Here's how the part is built. I have some questions about the finished solid (model axes, mm). Face numbers are marked on the shaded views. A direction names the side the tool comes from. Give positions to 0.01 mm unless a question says otherwise; leave off trailing zeros. Loops run counter-clockwise (first coordinate to the right, second up) from the corner with the lowest first, then second, coordinate; pieces in that order, holes last.
Q1. Suppose I cut it at B-B (z = 0). List the corners of the cut face in (x, y) for me.
Q2. Suppose I cut it at C-C (y = 7). List the corners of the cut face in (x, z) for me, and give its area (3 significant figures).
Q3. Suppose I cut it at D-D (y = 37). List the corners of the cut face in (x, z) for me, and give its area (3 significant figures).
Q4. I'm going to push flat-ended pins straight in: P1, Ø5, axis at y = 19, z = 3, coming from the +X side; P2, Ø6, axis at x = -1, y = 27.5, coming from the +Z side; P3, Ø2, axis at y = 16.5, z = -1.5, coming from the -X side. Where does each tip first touch, or does it pass through?
Q5. For the marked faces 1 and 2, which set-ups out of +Z, -Z, +X, -X, +Y, -Y let a thin tool reach every point of the face, with its end or its side?
Q6. Suppose I cut it at A-A (x = 0). List the corners of the cut face in (y, z) for me.
Q7. I need wall thicknesses on probe 1 along Y at (x, z) = (-5.75, 2); probe 2 along X at (y, z) = (27, -3); probe 3 along X at (y, z) = (12, 0.25). Which ranges of each line are inside material? Lowest first, please.
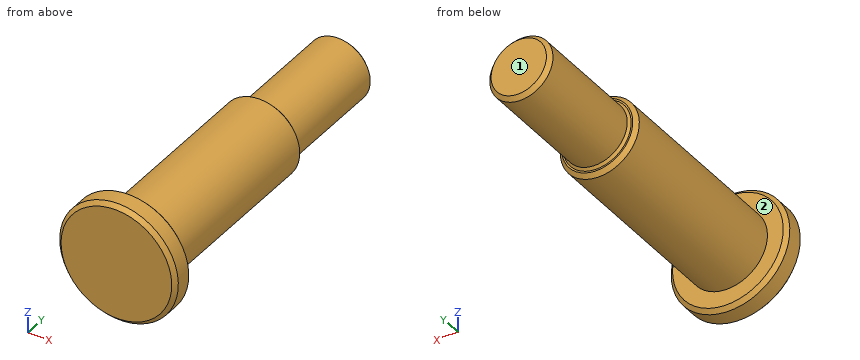
```python
from build123d import *

# Parameters (mm, degrees)
CHAMFER1_SIZE = 0.5
CHAMFER2_SIZE = 0.3


with BuildPart() as part:
    # Sketch1 → Revolve1 (revolve)
    with BuildSketch(Plane.XY, mode=Mode.PRIVATE) as revolve1_sk:
        Polygon((0, 0), (7.5, 0), (7.5, 3), (5, 3), (5, 28), (4, 28), (4, 43), (0, 43), align=None)
    revolve(revolve1_sk.sketch.rotate(Axis((0, 0, 0), (0, -1, 0)), 90), axis=Axis((0, 0, 0), (0, -1, 0)))

    # Chamfer1
    chamfer1_edges = [part.edges().sort_by_distance(p)[0] for p in [
        (0, 43, -4),
        (0, 28, -5),
        (0, 3, -7.5),
        (0, 0, -7.5),
    ]]
    chamfer(chamfer1_edges, length=CHAMFER1_SIZE)

    # Chamfer2
    chamfer2_edges = [part.edges().sort_by_distance(p)[0] for p in [
        (0, 28, -4),
    ]]
    chamfer(chamfer2_edges, length=CHAMFER2_SIZE)


solid = part.part
```
Solutions:
1. outline: (-7.5, 0.5) - (-7, 0) - (7, 0) - (7.5, 0.5) - (7.5, 2.5) - (7, 3) - (5, 3) - (5, 27.5) - (4.5, 28) - (4.3, 28) - (4, 28.3) - (4, 42.5) - (3.5, 43) - (-3.5, 43) - (-4, 42.5) - (-4, 28.3) - (-4.3, 28) - (-4.5, 28) - (-5, 27.5) - (-5, 3) - (-7, 3) - (-7.5, 2.5) - close
2. outline: circle Ø10 at (0, 0)
2. area: 78.5 mm2
3. outline: circle Ø8 at (0, 0)
3. area: 50.3 mm2
4. P1: stops at x = 4.97
4. P2: stops at z = 5
4. P3: stops at x = -4.97
5. face 1: +Z, -Z, +X, -X, +Y
5. face 2: +Y
6. outline: (0, -7) - (0.5, -7.5) - (2.5, -7.5) - (3, -7) - (3, -5) - (27.5, -5) - (28, -4.5) - (28, -4.3) - (28.3, -4) - (42.5, -4) - (43, -3.5) - (43, 3.5) - (42.5, 4) - (28.3, 4) - (28, 4.3) - (28, 4.5) - (27.5, 5) - (3, 5) - (3, 7) - (2.5, 7.5) - (0.5, 7.5) - (0, 7) - close
7. probe 1: y = 0 to 3
7. probe 2: x = -4 to 4
7. probe 3: x = -4.99 to 4.99
